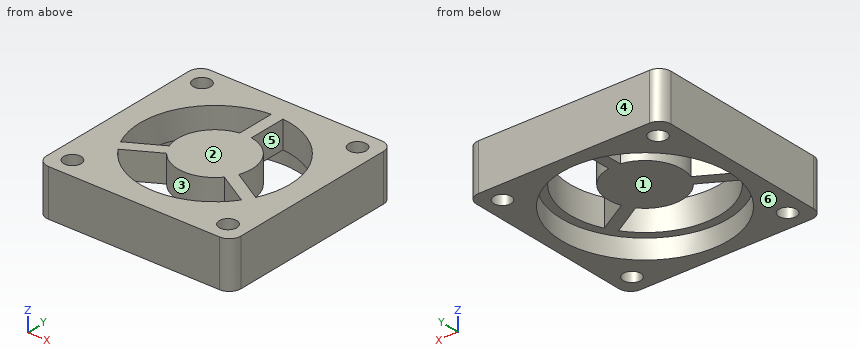
```python
from build123d import *

# Parameters (mm, degrees)
SKETCH1_R           = 2.25
BOSS_EXTRUDE1_DEPTH = 12
CUT_EXTRUDE1_DEPTH  = 12
SKETCH3_R           = 21.449558408
CUT_EXTRUDE2_DEPTH  = 5


with BuildPart() as part:
    # Sketch1 → Boss-Extrude1 (new body)
    with BuildSketch(Plane.XY):
        with BuildLine():
            Line((-22, 25), (22, 25))
            ThreePointArc((22, 25), (24.121320344, 24.121320344), (25, 22))
            Line((25, 22), (25, -22))
            ThreePointArc((25, -22), (24.121320344, -24.121320344), (22, -25))
            Line((22, -25), (-22, -25))
            ThreePointArc((-22, -25), (-24.121320344, -24.121320344), (-25, -22))
            Line((-25, -22), (-25, 22))
            ThreePointArc((-25, 22), (-24.121320344, 24.121320344), (-22, 25))
        make_face()
        with Locations((-20, 20)):
            Circle(SKETCH1_R, mode=Mode.SUBTRACT)
        with Locations((20, 20)):
            Circle(SKETCH1_R, mode=Mode.SUBTRACT)
        with Locations((20, -20)):
            Circle(SKETCH1_R, mode=Mode.SUBTRACT)
        with Locations((-20, -20)):
            Circle(SKETCH1_R, mode=Mode.SUBTRACT)
    extrude(amount=BOSS_EXTRUDE1_DEPTH)

    # Sketch2 → Cut-Extrude1 (cut)
    with BuildSketch(Plane.XY.offset(12)):
        with BuildLine():
            Line((-1.5, 19.188784117), (-1.5, 9.440713214))
            ThreePointArc((-1.5, 9.440713214), (-8.278453932, 4.779567606), (-8.925897474, -3.421318502))
            Line((-8.925897474, -3.421318502), (-17.367974513, -8.295353953))
            ThreePointArc((-17.367974513, -8.295353953), (-16.668670521, 9.623661412), (-1.5, 19.188784117))
        make_face()
        with BuildLine():
            Line((1.5, 19.188784117), (1.5, 9.440713214))
            ThreePointArc((1.5, 9.440713214), (8.278453932, 4.779567606), (8.925897474, -3.421318502))
            Line((8.925897474, -3.421318502), (17.367974513, -8.295353953))
            ThreePointArc((17.367974513, -8.295353953), (16.668670521, 9.623661412), (1.5, 19.188784117))
        make_face()
        with BuildLine():
            Line((15.867974513, -10.893430164), (7.425897474, -6.019394713))
            ThreePointArc((7.425897474, -6.019394713), (0, -9.559135212), (-7.425897474, -6.019394713))
            Line((-7.425897474, -6.019394713), (-15.867974513, -10.893430164))
            ThreePointArc((-15.867974513, -10.893430164), (0, -19.247322824), (15.867974513, -10.893430164))
        make_face()
    extrude(amount=-CUT_EXTRUDE1_DEPTH, mode=Mode.SUBTRACT)

    # Sketch3 → Cut-Extrude2 (cut)
    with BuildSketch(Plane(origin=(0, 0, 0), x_dir=(-1, 0, 0), z_dir=(0, 0, -1))):
        Circle(SKETCH3_R)
    extrude(amount=-CUT_EXTRUDE2_DEPTH, mode=Mode.SUBTRACT)


solid = part.part
```
Geometry check sheet. Reference: the model listing, model coordinates, mm. Face numbers are marked on the shaded views. A direction names the side the tool comes from. Give positions to 0.01 mm unless a question says otherwise; leave off trailing zeros. Loops run counter-clockwise (first coordinate to the right, second up) from the corner with the lowest first, then second, coordinate; pieces in that order, holes last. Notation, with made-up numbers: M 1.25,19.25 L 29.25,19.25 A19 cw 29.25,31.25 Z; hole C 26,52.25 d5. An arc over 180 degrees is marked long. Write item = value, one per line. Start each with the question number.
1. Section check A-A, the plane y = 0. Enter the section's corners in (x, z), plus the area to 3 significant figures.
2. Section check B-B, the plane x = 0. Enter the section's corners in (y, z), plus the area to 3 significant figures.
3. Thickness scan on probe 1 along Y at (x, z) = (20, 7); probe 2 along Y at (x, z) = (10, 7.25); probe 3 along Y at (x, z) = (0, 1.75). Record the ranges inside material, lowest first.
4. Section check C-C, the plane x = -5. Enter the section's corners in (y, z), plus the area to 3 significant figures.
5. Draft check along Y on the marked faces 4, 5 and 6. Enter one of: +Y half, -Y half, draft (parallel to the pull), parting line (faces both ways), or undercut.
6. Go/stop test with a flat-tipped pin: P1, Ø2.5, axis at x = 20, y = 20, coming from the -Z side. Record where the tip stops, or that it passes through.
7. Tool access check on the marked faces 1, 2 and 3. Record the directions out of +Z, -Z, +X, -X, +Y, -Y that give a thin tool (end or side, any length) a straight path to the whole face; none if there is none.
8. Section check D-D, the plane z = 2. Enter the section's corners in (x, y).
Values follow:
q1.outline = M -25,0 L -21.45,0 L -21.45,5 L -19.25,5 L -19.25,12 L -25,12 Z; M -9.56,5 L 9.56,5 L 9.56,12 L -9.56,12 Z; M 19.25,5 L 21.45,5 L 21.45,0 L 25,0 L 25,12 L 19.25,12 Z
q1.area = 250 mm^2
q2.outline = M -25,0 L -21.45,0 L -21.45,5 L -19.25,5 L -19.25,12 L -25,12 Z; M -9.56,5 L 21.45,5 L 21.45,0 L 25,0 L 25,12 L -9.56,12 Z
q2.area = 318 mm^2
q3.probe_1 = -25 to -22.25, -17.75 to 17.75, 22.25 to 25
q3.probe_2 = -25 to -16.45, -7.51 to -4.04, 16.45 to 25
q3.probe_3 = -25 to -21.45, 21.45 to 25
q4.outline = M -25,0 L -20.86,0 L -20.86,5 L -18.59,5 L -18.59,12 L -25,12 Z; M -8.15,5 L 8.15,5 L 8.15,12 L -8.15,12 Z; M 18.59,5 L 20.86,5 L 20.86,0 L 25,0 L 25,12 L 18.59,12 Z
q4.area = 245 mm^2
q5.face_4 = +Y half
q5.face_5 = undercut
q5.face_6 = draft
q6.P1 = through
q7.face_1 = -Z
q7.face_2 = +Z, +X, -X, +Y, -Y
q7.face_3 = +Z, -Z
q8.outline = M -25,-22 A3 ccw -22,-25 L 22,-25 A3 ccw 25,-22 L 25,22 A3 ccw 22,25 L -22,25 A3 ccw -25,22 Z; hole C -20,-20 d4.5; hole C -20,20 d4.5; hole C 0,0 d42.9; hole C 20,-20 d4.5; hole C 20,20 d4.5
